Geometry: final body of the model. Coordinates: model frame, mm. A direction names the side the tool comes from. Give positions to 0.01 mm unless a question says otherwise; leave off trailing zeros. Order: outer loops, then holes, each group sorted by start corner. A loop starts at its lowest first (then second) coordinate and runs counter-clockwise, first axis right, second up. Notation, with made-up numbers: (-0.75, -12) - (45.25, -12) arc R32 cw to (45.25, 17) - close; hole circle Ø5 at (31, 77). An arc over 180 degrees is marked (long way). Put each result on its own line as item: value. Start each with the question number.
1. First-contact query: P1, Ø2, axis at x = -0.5, z = 3.5, coming from the +Y side; P2, Ø1.3, axis at y = 0.5, z = 4, coming from the +X side; P3, Ø0.9, axis at x = 0, y = -3, coming from the +Z side. Flat tips, straight axial feed; report the tip coordinate or a pass-through.
2. Section B-B on x = 0. Return the cut outline in (y, z).
3. Section D-D on y = 2.75. Return the cut outline in (x, z), plus the area to 3 significant figures.
4. Section A-A on y = 1.25. Return the cut outline in (x, z).
5. Set-up query: faces 1 (the flat face through (-1.5, 0, 5)), 2 (the cylindrical face through (0, 4.5, 5.5)), 3 (the flat face through (0, -2, 5)), 4 (the flat face through (0, 0.5, 3)), 5 (the flat face through (2.5, 1.5, 0.5)). Return all of +Z, -Z, +X, -X, +Y, -Y with unobstructed straight access to the full face (end or side cutting, diameter ignored); none if empty.
6. Ray query, line 1 along Y through (x, z) = (-2.25, 0.65); line 2 along Y through (x, z) = (0, 5.6); line 3 along Z through (x, y) = (0.35, 1.75). Return the intervals inside material, ascending. Write a range as from..to.
7. Section C-C on x = 0.9. Return the cut outline in (y, z), plus the area to 3 significant figures.
8. Mould query, pull axis Z, two halves, no side actions, for faces 6 (the flat face through (0, 1, 1)), 7 (the flat face through (0, 0, 0)), 8 (the flat face through (1.5, 0, 5)). Classes: pulls with the +Z half, pulls with the -Z half, needs draft (parallel to the pull), parting line crosses it, or undercut.
from build123d import *

# Parameters (mm, degrees)
BASE_PLATE_DEPTH         = 1
WEB_SKETCH_W             = 3
WEB_SKETCH_H             = 1
WEB_DEPTH                = 4
LINK_PLATE_SKETCH_R      = 0.75
LINK_PLATE_DEPTH         = 1
WEB_ROOT_FILLET_R0_5_A_R = 0.5
WEB_ROOT_FILLET_R0_5_B_R = 0.5


with BuildPart() as part:
    # Base Plate Sketch → Base Plate (new body)
    with BuildSketch(Plane.XY):
        with BuildLine():
            Line((-3, 3.5), (-2, 3.5))
            ThreePointArc((-2, 3.5), (-1, 2.5), (-2, 1.5))
            Line((-2, 1.5), (-3, 1.5))
            Line((-3, 1.5), (-3, -1.5))
            Line((-3, -1.5), (-2, -1.5))
            ThreePointArc((-2, -1.5), (-1, -2.5), (-2, -3.5))
            Line((-2, -3.5), (-3, -3.5))
            Line((-3, -3.5), (-3, -4.5))
            Line((-3, -4.5), (3, -4.5))
            Line((3, -4.5), (3, -3.5))
            Line((3, -3.5), (2, -3.5))
            ThreePointArc((2, -3.5), (1, -2.5), (2, -1.5))
            Line((2, -1.5), (3, -1.5))
            Line((3, -1.5), (3, 1.5))
            Line((3, 1.5), (2, 1.5))
            ThreePointArc((2, 1.5), (1, 2.5), (2, 3.5))
            Line((2, 3.5), (3, 3.5))
            Line((3, 3.5), (3, 4.5))
            Line((3, 4.5), (-3, 4.5))
            Line((-3, 4.5), (-3, 3.5))
        make_face()
    extrude(amount=BASE_PLATE_DEPTH)

    # Web Sketch → Web (add)
    with BuildSketch(Plane.XY.offset(1)):
        Rectangle(WEB_SKETCH_W, WEB_SKETCH_H)
    extrude(amount=WEB_DEPTH)

    # Link Plate Sketch → Link Plate (add)
    with BuildSketch(Plane.XY.offset(5)):
        with BuildLine():
            Line((1.5, 3), (1.5, -3))
            ThreePointArc((1.5, -3), (0, -4.5), (-1.5, -3))
            Line((-1.5, -3), (-1.5, 3))
            ThreePointArc((-1.5, 3), (0, 4.5), (1.5, 3))
        make_face()
        with Locations((0, 3)):
            Circle(LINK_PLATE_SKETCH_R, mode=Mode.SUBTRACT)
        with Locations((0, -3)):
            Circle(LINK_PLATE_SKETCH_R, mode=Mode.SUBTRACT)
    extrude(amount=LINK_PLATE_DEPTH)

    # Web Root Fillet R0.5 A
    web_root_fillet_r0_5_a_edges = [part.edges().sort_by_distance(p)[0] for p in [
        (1.5, 0, 1),
    ]]
    fillet(web_root_fillet_r0_5_a_edges, radius=WEB_ROOT_FILLET_R0_5_A_R)

    # Web Root Fillet R0.5 B
    web_root_fillet_r0_5_b_edges = [part.edges().sort_by_distance(p)[0] for p in [
        (-1.5, 0, 1),
    ]]
    fillet(web_root_fillet_r0_5_b_edges, radius=WEB_ROOT_FILLET_R0_5_B_R)


solid = part.part
Resolved:
1. P1: y = 0.5
1. P2: x = 1.5
1. P3: z = 1
2. outline: (-4.5, 0) - (4.5, 0) - (4.5, 1) - (0.5, 1) - (0.5, 5) - (2.25, 5) - (2.25, 6) - (-2.25, 6) - (-2.25, 5) - (-0.5, 5) - (-0.5, 1) - (-4.5, 1) - close; (-4.5, 5) - (-3.75, 5) - (-3.75, 6) - (-4.5, 6) - close; (3.75, 5) - (4.5, 5) - (4.5, 6) - (3.75, 6) - close
3. outline: (-1.5, 5) - (-0.71, 5) - (-0.71, 6) - (-1.5, 6) - close; (-1.03, 0) - (1.03, 0) - (1.03, 1) - (-1.03, 1) - close; (0.71, 5) - (1.5, 5) - (1.5, 6) - (0.71, 6) - close
3. area: 3.65 mm^2
4. outline: (-3, 0) - (3, 0) - (3, 1) - (-3, 1) - close; (-1.5, 5) - (1.5, 5) - (1.5, 6) - (-1.5, 6) - close
5. face 1: +Z, -X, +Y, -Y
5. face 2: +Z, +Y
5. face 3: +X, -X, -Y
5. face 4: +X, -X, +Y
5. face 5: +Z, -Z, +X
6. line 1: -4.5..-3.5, -1.5..1.5, 3.5..4.5
6. line 2: -4.5..-3.75, -2.25..2.25, 3.75..4.5
6. line 3: 0..1, 5..6
7. outline: (-4.5, 0) - (4.5, 0) - (4.5, 1) - (0.5, 1) - (0.5, 5) - (4.2, 5) - (4.2, 6) - (-4.2, 6) - (-4.2, 5) - (-0.5, 5) - (-0.5, 1) - (-4.5, 1) - close
7. area: 21.4 mm^2
8. face 6: undercut
8. face 7: pulls with the -Z half
8. face 8: needs draft
